Geometry check sheet. Reference: the model listing, model coordinates, mm. Coordinates: 2 decimals unless noted, no trailing zeros. Write each loop counter-clockwise with the first axis right and the second up, starting at its lowest first coordinate (ties: lowest second). Pieces come first, ordered by that corner, then holes. Notation, with made-up numbers: (-34, 51) -> (-30, 51) arc R27 cw to (-30, 90) -> close; hole circle Ø4 at (4.25, -9). An arc over 180 degrees is marked (long way). Answer in a Markdown table with one row per item. Add a question column.
1. Mould release check, pull along Z, two halves, no side actions. Record for faces 1 (the cylindrical face through (1.802, -0.056, 5.723)), 2 (the flat face through (6, -4, 3)), 3 (the flat face through (-11.31, 0.06, 6.41)): pulls with the +Z half, pulls with the -Z half, needs draft (parallel to the pull), parting line crosses it, or undercut.
2. Depth check by flat-ended pin: P1, Ø1, axis at x = -9, y = -1, coming from the -Z side. Enter the tip coordinate at first touch or a pass-through.
3. Cross-section at A-A on y = -1. Record the cut outline in (x, z).
4. Scan lines: L1, parallel to X at y = -0.25, z = -5.5; L2, parallel to X at y = 1, z = -3; L3, parallel to Z at x = -4, y = 1.5. Record each from-to range of solid material in increasing order. Write a range as from..to.
```python
from build123d import *

# Parameters (mm, degrees)
HEX_PROFILE_SKETCH_R                  = 6
HEX_NUT_BODY_DEPTH                    = 4
CHAMFER_CIRCLE_SKETCH_OUTSIDE_W       = 163.26
CHAMFER_CIRCLE_SKETCH_OUTSIDE_H       = 159.238
CHAMFER_CIRCLE_SKETCH_OUTSIDE_R       = 13
TOP_CHAMFER_CUT_70DEG_DEPTH           = 22.408720964
TOP_CHAMFER_CUT_70DEG_DRAFT           = -70
BOTTOM_CHAMFER_MIRROR_COPY_1_SKETCH_W = 163.26
BOTTOM_CHAMFER_MIRROR_COPY_1_SKETCH_H = 159.238
BOTTOM_CHAMFER_MIRROR_COPY_1_SKETCH_R = 13
BOTTOM_CHAMFER_MIRROR_COPY_1_DEPTH    = 22.408720964
BOTTOM_CHAMFER_MIRROR_COPY_1_DRAFT    = -70


with BuildPart() as part:
    # Hex Profile Sketch → Hex Nut Body (new, symmetric)
    with BuildSketch(Plane(origin=(0, 0, 0), x_dir=(1, 0, 0), z_dir=(0, 1, 0))):
        Polygon((15.011106999, 0), (7.505553499, 13), (-7.505553499, 13), (-15.011106999, 0), (-7.505553499, -13), (7.505553499, -13), align=None)
        with Locations(Location((0, 0, 0), (0, 0, 270))):
            Circle(HEX_PROFILE_SKETCH_R, mode=Mode.SUBTRACT)
    extrude(amount=HEX_NUT_BODY_DEPTH, both=True)


with BuildPart() as top_chamfer_cut_70deg_tool:
    # Chamfer Circle Sketch outside → Top Chamfer Cut 70deg (with draft: the straight prism first)
    with BuildSketch(Plane(origin=(0, 4, 0), x_dir=(1, 0, 0), z_dir=(0, 1, 0))):
        Rectangle(CHAMFER_CIRCLE_SKETCH_OUTSIDE_W, CHAMFER_CIRCLE_SKETCH_OUTSIDE_H)
        Circle(CHAMFER_CIRCLE_SKETCH_OUTSIDE_R, mode=Mode.SUBTRACT)
    extrude(amount=-TOP_CHAMFER_CUT_70DEG_DEPTH)
    # Top Chamfer Cut 70deg: the draft: its side faces are tilted about the plane it starts from
    top_chamfer_cut_70deg_sides = [top_chamfer_cut_70deg_tool.faces().sort_by_distance(p)[0] for p in [
        (0, -7.204360482, 79.619),
        (81.63, -7.204360482, 0),
        (0, -7.204360482, -79.619),
        (-81.63, -7.204360482, 0),
        (-13, -7.204360482, 0),
    ]]
    draft(top_chamfer_cut_70deg_sides, Plane(origin=(0, 4, 0), x_dir=(1, 0, 0), z_dir=(0, 1, 0)), TOP_CHAMFER_CUT_70DEG_DRAFT)


with BuildPart() as part_1:
    add(part.part)

    # Top Chamfer Cut 70deg: cut by top_chamfer_cut_70deg_tool
    add(top_chamfer_cut_70deg_tool.part, mode=Mode.SUBTRACT)


with BuildPart() as bottom_chamfer_mirror_copy_1_tool:
    # Bottom Chamfer Mirror copy 1 sketch → Bottom Chamfer Mirror copy 1 (with draft: the straight prism first)
    with BuildSketch(Plane.XZ.offset(4)):
        Rectangle(BOTTOM_CHAMFER_MIRROR_COPY_1_SKETCH_W, BOTTOM_CHAMFER_MIRROR_COPY_1_SKETCH_H)
        Circle(BOTTOM_CHAMFER_MIRROR_COPY_1_SKETCH_R, mode=Mode.SUBTRACT)
    extrude(amount=-BOTTOM_CHAMFER_MIRROR_COPY_1_DEPTH)
    # Bottom Chamfer Mirror copy 1: the draft: its side faces are tilted about the plane it starts from
    bottom_chamfer_mirror_copy_1_sides = [bottom_chamfer_mirror_copy_1_tool.faces().sort_by_distance(p)[0] for p in [
        (0, 7.204360482, 79.619),
        (81.63, 7.204360482, 0),
        (0, 7.204360482, -79.619),
        (-81.63, 7.204360482, 0),
        (-13, 7.204360482, 0),
    ]]
    draft(bottom_chamfer_mirror_copy_1_sides, Plane.XZ.offset(4), BOTTOM_CHAMFER_MIRROR_COPY_1_DRAFT)


with BuildPart() as part_2:
    add(part_1.part)

    # Bottom Chamfer Mirror copy 1: cut by bottom_chamfer_mirror_copy_1_tool
    add(bottom_chamfer_mirror_copy_1_tool.part, mode=Mode.SUBTRACT)


solid = part_2.part
```
Results found:
| question | item | result |
|---|---|---|
| 1 | face 1 | undercut |
| 1 | face 2 | needs draft |
| 1 | face 3 | pulls with the +Z half |
| 2 | P1 | stops at z = -11.28 |
| 3 | outline | (-15.01, 0) -> (-7.51, -13) -> (7.51, -13) -> (15.01, 0) -> (7.51, 13) -> (-7.51, 13) -> close; hole circle Ø12 at (0, 0) |
| 4 | L1 | x = -11.84..-2.4, 2.4..11.84 |
| 4 | L2 | x = -13.28..-5.2, 5.2..13.28 |
| 4 | L3 | z = -13..-4.47, 4.47..13 |
